```python
from build123d import *

# Parameters (mm, degrees)
SKETCH1_R           = 30
BOSS_EXTRUDE1_DEPTH = 5
SKETCH2_R           = 2.5
CUT_EXTRUDE1_DEPTH  = 5
SKETCH3_R           = 5
BOSS_EXTRUDE2_DEPTH = 18
SKETCH4_R           = 12.5
BOSS_EXTRUDE3_DEPTH = 10
FILLET1_R           = 2


with BuildPart() as part:
    # Sketch1 → Boss-Extrude1 (new body)
    with BuildSketch(Plane.XY):
        Circle(SKETCH1_R)
    extrude(amount=BOSS_EXTRUDE1_DEPTH)

    # Sketch2 → Cut-Extrude1 (cut)
    with BuildSketch(Plane.XY.offset(5)):
        Circle(SKETCH2_R)
    extrude(amount=-CUT_EXTRUDE1_DEPTH, mode=Mode.SUBTRACT)

    # Sketch3 → Boss-Extrude2 (add)
    with BuildSketch(Plane.XY.offset(5)):
        with Locations((20.816087355, 8.573414189)):
            Circle(SKETCH3_R)
    extrude(amount=BOSS_EXTRUDE2_DEPTH)

    # Sketch4 → Boss-Extrude3 (add)
    with BuildSketch(Plane.XY.offset(23)):
        with Locations((20.816087355, 8.573414189)):
            Circle(SKETCH4_R)
    extrude(amount=BOSS_EXTRUDE3_DEPTH)

    # Fillet1
    fillet1_edges = [part.edges().sort_by_distance(p)[0] for p in [
        (8.316087355, 8.573414189, 23),
        (8.316087355, 8.573414189, 33),
    ]]
    fillet(fillet1_edges, radius=FILLET1_R)


solid = part.part
```
Geometry check sheet. Reference: the model listing, model coordinates, mm. A direction names the side the tool comes from. Round coordinates to 2 decimals unless told otherwise and drop trailing zeros. Loops run counter-clockwise (first coordinate to the right, second up) from the corner with the lowest first, then second, coordinate; pieces in that order, holes last. Notation, with made-up numbers: M 8.25,-30 L 55.25,-30 A27 ccw 55.25,6 Z; hole C 66.5,43.5 d9. An arc over 180 degrees is marked long. Return JSON: item names as keys, results as strings. Group by question number.
(1) Section check D-D, the plane y = -19.5. Enter the section's corners in (x, z).
(2) Mould release check, pull along X, two halves, no side actions. Record for faces 1 (the face through (32.363, 3.786, 27.958)), 2 (the face through (-0.54, -2.44, 2.54)), 3 (the face through (18, 4, 23)): pulls with the +X half, pulls with the -X half, needs draft (parallel to the pull), parting line crosses it, or undercut.
(3) Section check C-C, the plane z = 21. Enter the section's corners in (x, y).
(4) Scan lines: line 1 along Y through (x, z) = (0, 3.8); line 2 along Z through (x, y) = (20, 16.5); line 3 along Z through (x, y) = (13, -10). Record each from-to range of solid material in increasing order. Write a range as [from, to].
(5) Set-up check for faces 4 (the face through (25.585, 10.075, 13.874)), 5 (the face through (21, 9, 33)): record each of +Z, -Z, +X, -X, +Y, -Y from which the full face is reachable in a straight line by a thin tool's end or side.
(6) Section check A-A, the plane x = 0. Enter the section's corners in (y, z), and give its area (3 significant figures).
(7) Section check B-B, the plane y = 0. Give the number of separate pieces and of enclosed holes in the cut face, and give its area (3 significant figures).
(8) Go/stop test with flat-tipped pins: pin 1 (8 mm diameter, centred on x = 4, y = -6, fed in from +Z); pin 2 (3 mm diameter, centred on x = 21, z = 19.5, fed in from +Y); pin 3 (1.5 mm diameter, centred on x = 15.5, z = 8.5, fed in from +Y). Record where each tip stops, or that it passes through.
Data:
{
 "1": {"outline": "M -22.8,0 L 22.8,0 L 22.8,5 L -22.8,5 Z"},
 "2": {"face 1": "parting line crosses it", "face 2": "undercut", "face 3": "needs draft"},
 "3": {"outline": "C 20.82,8.57 d10"},
 "4": {"line 1": "[-30, -2.5], [2.5, 30]", "line 2": "[0, 5], [23, 33]", "line 3": "[0, 5]"},
 "5": {"face 4": "none", "face 5": "+Z, +X, -X, +Y, -Y"},
 "6": {"outline": "M -30,0 L -2.5,0 L -2.5,5 L -30,5 Z; M 2.5,0 L 30,0 L 30,5 L 2.5,5 Z", "area": "275 mm²"},
 "7": {"separate pieces": "3", "enclosed holes": "0", "area": "452 mm²"},
 "8": {"pin 1": "z = 5", "pin 2": "y = 13.57", "pin 3": "y = 10.61"}
}
